Input: part model. Units: mm. Frame: model coordinates. Coordinates: 2 decimals unless noted, no trailing zeros. Loops run counter-clockwise (first coordinate to the right, second up) from the corner with the lowest first, then second, coordinate; pieces in that order, holes last.
```python
from build123d import *

# Parameters (mm, degrees)
EXTRUDE_1_DEPTH = 600


with BuildPart() as part:
    # 草图1 → 凸台-拉伸1 (new body)
    with BuildSketch(Plane.XY.offset(-300)):
        Polygon((-10, -12.5), (-14, -12.5), (-14, -45.5), (11, -45.5), (11, -15.5), (-10, -15.5), align=None)
    extrude(amount=-EXTRUDE_1_DEPTH)


solid = part.part
```
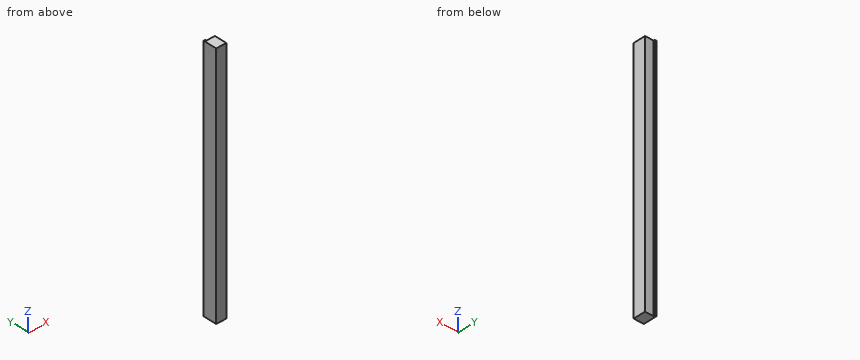
Item 1: Line query: L1, parallel to Y at x = -7.5, z = -442. Output: solid intervals per line, ascending.
Result:
L1: y = -45.5 to -15.5
Item 2: Section query B-B (x = -3). Output: boundary loops of the cut face in (y, z), then the cut area to 3 significant figures.
Result:
outline: (-45.5, -900) - (-15.5, -900) - (-15.5, -300) - (-45.5, -300) - close
area: 18,000 mm2
Item 3: Section query A-A (z = -563.5). Output: boundary loops of the cut face in (x, y), then the cut area to 3 significant figures.
Result:
outline: (-14, -45.5) - (11, -45.5) - (11, -15.5) - (-10, -15.5) - (-10, -12.5) - (-14, -12.5) - close
area: 762 mm2
Item 4: Contact query for flat-ended pins moving along their axis: P1, Ø1, axis at x = -8, z = -683.5, coming from the +Y side; P2, Ø2.5, axis at y = -14.5, z = -475, coming from the +X side. Output: stop coordinate, or through.
Result:
P1: stops at y = -15.5
P2: stops at x = 11
